CAD build for the part. Positions are in the model's coordinates, mm. A direction names the side the tool comes from. Round coordinates to 2 decimals unless told otherwise and drop trailing zeros. Order: outer loops, then holes, each group sorted by start corner. A loop starts at its lowest first (then second) coordinate and runs counter-clockwise, first axis right, second up. Notation, with made-up numbers: (30.5, -14.5) - (34.5, -14.5) arc R34 cw to (34.5, 17.5) - close; hole circle Ø2 at (89, -38.5). An arc over 180 degrees is marked (long way). Write item = value, one per line.
from build123d import *

# Parameters (mm, degrees)
SKETCH1_W             = 20
SKETCH1_H             = 55
BOSS_EXTRUDE1_DEPTH   = 20
SKETCH2_W             = 9
SKETCH2_H             = 55
CUT_EXTRUDE1_DEPTH    = 2
M3_TAPPED_HOLE1_D     = 2.5
M3_TAPPED_HOLE1_DEPTH = 7.5
M3_TAPPED_HOLE1_TIP   = 0.751075774
M4_TAPPED_HOLE1_D     = 3.3
M4_TAPPED_HOLE1_DEPTH = 10.1
M4_TAPPED_HOLE1_TIP   = 0.991420021
M5_TAPPED_HOLE1_D     = 4.2
M5_TAPPED_HOLE1_DEPTH = 12.4
M5_TAPPED_HOLE1_TIP   = 1.2618073
CHAMFER1_SIZE         = 1


with BuildPart() as part:
    # Sketch1 → Boss-Extrude1 (new body)
    with BuildSketch(Plane.XY):
        Rectangle(SKETCH1_W, SKETCH1_H)
    extrude(amount=BOSS_EXTRUDE1_DEPTH)

    # Sketch2 → Cut-Extrude1 (cut)
    with BuildSketch(Plane.XY.offset(20)):
        Rectangle(SKETCH2_W, SKETCH2_H)
    extrude(amount=-CUT_EXTRUDE1_DEPTH, mode=Mode.SUBTRACT)

    # M3 Tapped Hole1
    with Locations(Plane.XY.offset(18)):
        with Locations((0, 20), (0, 0), (0, -20)):
            Hole(M3_TAPPED_HOLE1_D / 2, depth=M3_TAPPED_HOLE1_DEPTH)
            with Locations((0, 0, -(M3_TAPPED_HOLE1_DEPTH + M3_TAPPED_HOLE1_TIP / 2))):  # 118° drill point
                Cone(0, M3_TAPPED_HOLE1_D / 2, M3_TAPPED_HOLE1_TIP, mode=Mode.SUBTRACT)

    # M4 Tapped Hole1
    with Locations(Plane(origin=(0, -27.5, 0), x_dir=(-1, 0, 0), z_dir=(0, -1, 0))):
        with Locations((0, -13), (0, -5.5)):
            Hole(M4_TAPPED_HOLE1_D / 2, depth=M4_TAPPED_HOLE1_DEPTH)
            with Locations((0, 0, -(M4_TAPPED_HOLE1_DEPTH + M4_TAPPED_HOLE1_TIP / 2))):  # 118° drill point
                Cone(0, M4_TAPPED_HOLE1_D / 2, M4_TAPPED_HOLE1_TIP, mode=Mode.SUBTRACT)

    # M5 Tapped Hole1
    with Locations(Plane(origin=(0, 0, 0), x_dir=(-1, 0, 0), z_dir=(0, 0, -1))):
        with Locations((0, 20), (0, -20)):
            Hole(M5_TAPPED_HOLE1_D / 2, depth=M5_TAPPED_HOLE1_DEPTH)
            with Locations((0, 0, -(M5_TAPPED_HOLE1_DEPTH + M5_TAPPED_HOLE1_TIP / 2))):  # 118° drill point
                Cone(0, M5_TAPPED_HOLE1_D / 2, M5_TAPPED_HOLE1_TIP, mode=Mode.SUBTRACT)

    # Chamfer1
    chamfer1_edges = [part.edges().sort_by_distance(p)[0] for p in [
        (-10, 0, 20),
        (10, 0, 20),
        (0, -27.5, 0),
        (-10, 0, 0),
        (0, 27.5, 0),
        (10, 0, 0),
        (10, -27.5, 10),
        (-10, -27.5, 10),
        (-10, 27.5, 10),
        (10, 27.5, 10),
    ]]
    chamfer(chamfer1_edges, length=CHAMFER1_SIZE)


solid = part.part
(1) Pull direction X, two halves, no side cores. Call faces 1 (the cylindrical face through (-0.4, -22.4, 14.6)), 2 (the flat face through (9.5, 27, 10.4)), 3 (the flat face through (-9.5, -0.4, 0.5)): released by +X, released by -X, zero draft, split by the parting line, or undercut.
Solved:
face_1 = undercut
face_2 = released by +X
face_3 = released by -X
(2) Probe line 1 along Z through (x, y) = (0, -17.65); line 2 along Y through (x, z) = (0, 8.25); line 3 along Z through (x, y) = (1, -22.5). List the from-to ranges inside material, lowest first.
Solved:
line_1 = 0 to 3.85, 7.15 to 11.35, 14.65 to 18
line_2 = -27.5 to -22.1, -17.9 to 17.9, 22.1 to 27.5
line_3 = 0 to 4.19, 6.81 to 11.69, 14.31 to 18
(3) Band-saw the part on B-B on z = 18.5. List the corners of the cut face in (x, y).
Solved:
outline = (-10, -26.5) - (-9, -27.5) - (-4.5, -27.5) - (-4.5, 27.5) - (-9, 27.5) - (-10, 26.5) - close; (4.5, -27.5) - (9, -27.5) - (10, -26.5) - (10, 26.5) - (9, 27.5) - (4.5, 27.5) - close
(4) Band-saw the part on C-C on y = 7.5. List the corners of the cut face in (x, z).
Solved:
outline = (-10, 1) - (-9, 0) - (9, 0) - (10, 1) - (10, 19) - (9, 20) - (4.5, 20) - (4.5, 18) - (-4.5, 18) - (-4.5, 20) - (-9, 20) - (-10, 19) - close
(5) Band-saw the part on D-D on y = -20. List the corners of the cut face in (x, z), plus the area to 3 significant figures.
Solved:
outline = (-10, 1) - (-9, 0) - (-2.1, 0) - (-2.1, 12.4) - (-1.62, 12.69) arc R1.65 cw to (-1.25, 14.08) - (-1.25, 18) - (-4.5, 18) - (-4.5, 20) - (-9, 20) - (-10, 19) - close; (1.25, 14.08) arc R1.65 cw to (1.62, 12.69) - (2.1, 12.4) - (2.1, 0) - (9, 0) - (10, 1) - (10, 19) - (9, 20) - (4.5, 20) - (4.5, 18) - (1.25, 18) - close
area = 313 mm²
(6) Tool access for faces 4 (the cylindrical face through (0.27, -1.22, 14.2)), 5 (the cylindrical face through (1.13, 21.77, 6.29)), 6 (the flat face through (-9.5, -0.4, 19.5)), 7 (the flat face through (-4.5, 0, 19)), 8 (the flat face through (-9.3, 26.9, 0.7)): list every direction of +Z, -Z, +X, -X, +Y, -Y with a clear straight run to the whole face (end or side of a thin tool).
Solved:
face_4 = +Z
face_5 = -Z
face_6 = +Z, -X, +Y, -Y
face_7 = +Z, +Y, -Y
face_8 = -Z, -X, +Y
(7) Band-saw the part on A-A on y = 20. List the corners of the cut face in (x, z), plus the area to 3 significant figures.
Solved:
outline = (-10, 1) - (-9, 0) - (-2.1, 0) - (-2.1, 12.4) - (-1.25, 12.91) - (-1.25, 18) - (-4.5, 18) - (-4.5, 20) - (-9, 20) - (-10, 19) - close; (1.25, 12.91) - (2.1, 12.4) - (2.1, 0) - (9, 0) - (10, 1) - (10, 19) - (9, 20) - (4.5, 20) - (4.5, 18) - (1.25, 18) - close
area = 313 mm²
(8) Drop flat-ended pins along their axis: pin 1 (3 mm diameter, centred on x = 0, z = 13, fed in from -Y); pin 2 (2 mm diameter, centred on y = -6.5, z = 19.5, fed in from -X); pin 3 (7 mm diameter, centred on x = -0.5, y = 13.5, fed in from +Z); pin 4 (3.5 mm diameter, centred on x = 0, y = 20, fed in from -Z). Give the stop position or say it passes through.
Solved:
pin_1 = -17.31
pin_2 = -10
pin_3 = 18
pin_4 = 12.61
